```python
from build123d import *

# Parameters (mm, degrees)
BOSS_EXTRUDE1_DEPTH     = 5
BOSS_EXTRUDE2_DEPTH     = 10
CUT_EXTRUDE1_DEPTH      = 27.946503772
CUT_EXTRUDE1_DEPTH_BACK = 27.946503772
SKETCH3_R               = 2
CUT_EXTRUDE2_DEPTH      = 34.102948638
CUT_EXTRUDE2_DEPTH_BACK = 34.102948638
SKETCH4_R               = 1.5


with BuildPart() as part:
    # Sketch1 → Boss-Extrude1 (new body)
    with BuildSketch(Plane(origin=(0, 0, 0), x_dir=(1, 0, 0), z_dir=(0, 1, 0))):
        Polygon((0, 0), (-23, 0), (-23, 14.105675379), (-10.009618943, 21.605675379), (-1.863192499, 17.780007308), (0, 10), align=None)
    extrude(amount=BOSS_EXTRUDE1_DEPTH)

    # Sketch2 → Boss-Extrude2 (add)
    with BuildSketch(Plane(origin=(0, 5, 0), x_dir=(1, 0, 0), z_dir=(0, 1, 0))):
        Polygon((-22, 12.373624571), (-9.009618943, 19.873624571), (-10.009618943, 21.605675379), (-23, 14.105675379), align=None)
    extrude(amount=BOSS_EXTRUDE2_DEPTH)

    # Sketch3 → Cut-Extrude1 (cut, two sides: drawn at the far end of the back side and taken through both)
    with BuildSketch(Plane(origin=(-10.857936608, 0, -18.80649787), x_dir=(0.8660254037844384, 0, -0.5000000000000004), z_dir=(0.5000000000000004, 0, 0.8660254037844384)).offset(-CUT_EXTRUDE1_DEPTH_BACK)):
        with Locations((-9.365746598, 10)):
            Circle(SKETCH3_R)
        with Locations((-1.365746598, 10)):
            Circle(SKETCH3_R)
    extrude(amount=CUT_EXTRUDE1_DEPTH + CUT_EXTRUDE1_DEPTH_BACK, mode=Mode.SUBTRACT)

    # Sketch4 → Cut-Extrude2 (cut, two sides: drawn at the far end of the back side and taken through both)
    with BuildSketch(Plane(origin=(0, 5, 0), x_dir=(1, 0, 0), z_dir=(0, 1, 0)).offset(-CUT_EXTRUDE2_DEPTH_BACK)):
        with Locations(Location((-16.5, 5, 0), (0, 0, 270))):
            Circle(SKETCH4_R)
        with Locations(Location((-6.5, 5, 0), (0, 0, 270))):
            Circle(SKETCH4_R)
    extrude(amount=CUT_EXTRUDE2_DEPTH + CUT_EXTRUDE2_DEPTH_BACK, mode=Mode.SUBTRACT)


solid = part.part
```
Geometry: final body of the model. Coordinates: model frame, mm. A direction names the side the tool comes from. Coordinates: 2 decimals unless noted, no trailing zeros. Order: outer loops, then holes, each group sorted by start corner. A loop starts at its lowest first (then second) coordinate and runs counter-clockwise, first axis right, second up. Notation, with made-up numbers: (70.5, 47.5) - (91.5, 47.5) arc R30 ccw to (91.5, 77.5) - close; hole circle Ø2 at (-0.75, 31). An arc over 180 degrees is marked (long way). Return JSON: item names as keys, results as strings. Group by question number.
1. Pin query (flat end, axial travel): pin 1 (3 mm diameter, centred on x = -17, y = 11, fed in from -Z); pin 2 (1 mm diameter, centred on x = -18, z = -6.5, fed in from +Y); pin 3 (3 mm diameter, centred on y = 3.5, z = -19, fed in from -X); pin 4 (2.5 mm diameter, centred on x = -6.5, z = -5, fed in from +Y). Return the tip coordinate at first contact, or that it passes through.
2. Material intervals for line 1 along X through (y, z) = (2.9, -5); line 2 along Y through (x, z) = (-15.5, -14); line 3 along Z through (x, y) = (-6.5, 1.95), sorted ascending. Write a range as [from, to].
3. Cut plane B-B (y = 2.5). Output: boundary loops of the cut face in (x, z), plus the area to 3 significant figures.
4. Pull-direction query (X, two-part tool) for faces 4 (the face through (-12.773, 11.983, -18.872)), 5 (the face through (-11, 5, -9)), 6 (the face through (-0.945, 2.465, -13.944)); classes: pulls with the +X half, pulls with the -X half, needs draft (parallel to the pull), parting line crosses it, or undercut.
5. Cut plane A-A (x = -6.5). Output: boundary loops of the cut face in (y, z), plus the area to 3 significant figures.
6. Cut plane C-C (y = 10.5). Output: boundary loops of the cut face in (x, z), plus the area to 3 significant figures.
7. Set-up query: faces 1 (the face through (-15.6, 9.93, -16.07)), 2 (the face through (-9.503, 9.93, -20.728)), 3 (the face through (-22.507, 9.93, -13.252)). Return all of +Z, -Z, +X, -X, +Y, -Y with unobstructed straight access to the full face (end or side cutting, diameter ignored); none if empty.
8. Cut plane D-D (z = -7.75). Output: boundary loops of the cut face in (x, y).
Resolved:
{
 "1": {"pin 1": "stops at z = -18.44", "pin 2": "stops at y = 5", "pin 3": "stops at x = -17.12", "pin 4": "passes through"},
 "2": {"line 1": "x = [-23, -18], [-15, -8], [-5, 0]", "line 2": "y = [0, 5]", "line 3": "z = [-19.96, -6.5], [-3.5, 0]"},
 "3": {"outline": "(-23, -14.11) - (-10.01, -21.61) - (-1.86, -17.78) - (0, -10) - (0, 0) - (-23, 0) - close; hole circle Ø3 at (-16.5, -5); hole circle Ø3 at (-6.5, -5)", "area": "404 mm²"},
 "4": {"face 4": "undercut", "face 5": "needs draft", "face 6": "pulls with the +X half"},
 "5": {"outline": "(0, -19.96) - (5, -19.96) - (5, -6.5) - (0, -6.5) - close; (0, -3.5) - (5, -3.5) - (5, 0) - (0, 0) - close", "area": "84.8 mm²"},
 "6": {"outline": "(-23, -14.11) - (-21.65, -14.89) - (-20.65, -13.16) - (-22, -12.37) - close; (-18.29, -16.82) - (-14.72, -18.89) - (-13.72, -17.16) - (-17.29, -15.09) - close; (-11.36, -20.82) - (-10.01, -21.61) - (-9.01, -19.87) - (-10.36, -19.09) - close", "area": "14.5 mm²"},
 "7": {"face 1": "+Z, +X, +Y", "face 2": "-Z, +X, +Y", "face 3": "+Z, -X, +Y"},
 "8": {"outline": "(-23, 0) - (0, 0) - (0, 5) - (-23, 5) - close"}
}
